Build history of the part. All positions in model axes, mm. Face numbers are marked on the shaded views. A direction names the side the tool comes from. Give positions to 0.01 mm unless a question says otherwise; leave off trailing zeros. Loops run counter-clockwise (first coordinate to the right, second up) from the corner with the lowest first, then second, coordinate; pieces in that order, holes last. Notation, with made-up numbers: (72.25, 57) -> (107.25, 57) arc R15 ccw to (107.25, 69) -> close; hole circle Ø7 at (-26, 43.5). An arc over 180 degrees is marked (long way). Answer as a JSON object with one key per item and string values. Group by question number.
Q1. Band-saw the part on B-B, the plane y = -133.5. Write the cut outline in (x, z).
Q2. Two-plate mould, pull along Y, no slides. Class the marked faces 4, 5, 6 and 7: pulls with the +Y half, pulls with the -Y half, needs draft (parallel to the pull), parting line crosses it, or undercut.
Q3. Tool access for the marked faces 1, 2 and 3: list every direction of +Z, -Z, +X, -X, +Y, -Y with a clear straight run to the whole face (end or side of a thin tool).
Q4. Drop flat-ended pins along their axis: pin 1 (16.5 mm diameter, centred on x = -8, y = 127.5, fed in from -Z); pin 2 (15.5 mm diameter, centred on x = -20, y = -64, fed in from +Z); pin 3 (1 mm diameter, centred on x = 54.5, z = 6, fed in from +Y); pin 4 (1 mm diameter, centred on x = 2.5, y = -122, fed in from -Z). Give the stop position or say it passes through.
Q5. Wall check: probe 1 along X at (y, z) = (-64, -37); probe 2 along X at (y, z) = (-64, -16.5); probe 3 along Y at (x, z) = (-20, 1). Give the ranges that are in metal, low to high. Write a range as from..to.
Q6. Band-saw the part on D-D, the plane y = 106.5. Write the cut outline in (x, z), plus the area to 3 significant figures.
Q7. Band-saw the part on A-A, the plane x = -32. Write the cut outline in (y, z).
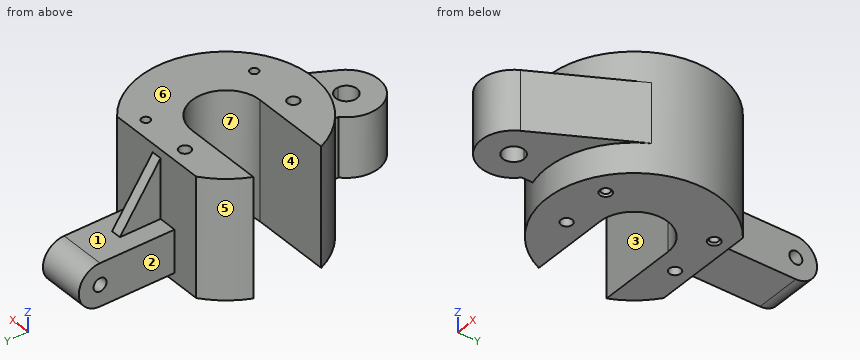
from build123d import *

# Parameters (mm, degrees)
CLAMP_BODY_PROFILE_R      = 5
CLAMP_BODY_PROFILE_R_2    = 6.75
CLAMP_BODY_DEPTH          = 70
TOP_LUG_AND_RIB_PROFILE_R = 7.668976578
TOP_LUG_DEPTH             = 27.5
GUSSET_RIB_DEPTH          = 6
BOTTOM_LUG_DEPTH          = 35
EDGE_CHAMFER_2X45_SIZE    = 2


with BuildPart() as part:
    # Clamp Body Profile → Clamp Body (new, symmetric)
    with BuildSketch(Plane.XY):
        with BuildLine():
            Line((0, -40), (-93.829632846, -40))
            ThreePointArc((-93.829632846, -40), (63.213972543, -80.04994488), (60.663003552, 82))
            Line((60.663003552, 82), (-60.663003552, 82))
            ThreePointArc((-60.663003552, 82), (-80.04994488, 63.213972543), (-93.829632846, 40))
            Line((-93.829632846, 40), (0, 40))
            ThreePointArc((0, 40), (40, 0), (0, -40))
        make_face()
        with Locations((39.991638522, 64)):
            Circle(CLAMP_BODY_PROFILE_R, mode=Mode.SUBTRACT)
        with Locations((-20, 64)):
            Circle(CLAMP_BODY_PROFILE_R_2, mode=Mode.SUBTRACT)
        with Locations(Location((39.991638522, -64, 0), (0, 0, 180))):
            Circle(CLAMP_BODY_PROFILE_R, mode=Mode.SUBTRACT)
        with Locations(Location((-20, -64, 0), (0, 0, 180))):
            Circle(CLAMP_BODY_PROFILE_R_2, mode=Mode.SUBTRACT)
    extrude(amount=CLAMP_BODY_DEPTH, both=True)

    # Top Lug and Rib Profile → Top Lug (add, symmetric)
    with BuildSketch(Plane(origin=(0, 0, 0), x_dir=(0, 0, -1), z_dir=(1, 0, 0))):
        with BuildLine():
            Line((60, 82), (60, 170))
            ThreePointArc((60, 170), (35, 195), (10, 170))
            Line((10, 170), (10, 130))
            Line((10, 130), (10, 82))
            Line((10, 82), (60, 82))
        make_face()
        with Locations((35, 170)):
            Circle(TOP_LUG_AND_RIB_PROFILE_R, mode=Mode.SUBTRACT)
    extrude(amount=TOP_LUG_DEPTH, both=True)

    # Sketch6_3 → Gusset Rib (add, symmetric)
    with BuildSketch(Plane(origin=(0, 0, 0), x_dir=(0, 0, -1), z_dir=(1, 0, 0))):
        Polygon((-60, 82), (10, 82), (10, 130), align=None)
    extrude(amount=GUSSET_RIB_DEPTH, both=True)

    # Bottom Lug Profile → Bottom Lug (add, symmetric)
    with BuildSketch(Plane.XY):
        with BuildLine():
            ThreePointArc((-27.5, -111.367680386), (-26.163106523, -169.703640044), (30.991702616, -157.947821666))
            Line((30.991702616, -157.947821666), (89.874157687, -48.235213071))
            ThreePointArc((89.874157687, -48.235213071), (51.583370989, -87.995203491), (-1.814745181, -101.983855094))
            ThreePointArc((-1.814745181, -101.983855094), (-2.152772572, -101.979344048), (-2.490826719, -101.977840326))
            Line((-2.490826719, -101.977840326), (-2.490826719, -101.969582633))
            ThreePointArc((-2.490826719, -101.969582633), (-15.1119726, -100.87431925), (-27.5, -98.222960656))
            Line((-27.5, -98.222960656), (-27.5, -111.367680386))
        make_face()
        with BuildLine():
            ThreePointArc((10.009173281, -139.977840326), (-11.329661484, -148.816675091), (-2.490826719, -127.477840326))
            ThreePointArc((-2.490826719, -127.477840326), (6.348008046, -131.139005561), (10.009173281, -139.977840326))
        make_face(mode=Mode.SUBTRACT)
    extrude(amount=BOTTOM_LUG_DEPTH, both=True)

    # Edge Chamfer 2x45
    edge_chamfer_2x45_edges = [part.edges().sort_by_distance(p)[0] for p in [
        (34.991638522, 64, -70),
        (44.991638522, -64, -70),
    ]]
    chamfer(edge_chamfer_2x45_edges, length=EDGE_CHAMFER_2X45_SIZE)


solid = part.part
Worked answers:
{
 "1": {"outline": "(-39.93, -35) -> (-13.18, -35) -> (-13.18, 35) -> (-39.93, 35) -> close; (8.2, -35) -> (44.11, -35) -> (44.11, 35) -> (8.2, 35) -> close"},
 "2": {"face 4": "undercut", "face 5": "pulls with the +Y half", "face 6": "needs draft", "face 7": "undercut"},
 "3": {"face 1": "+Z, +Y", "face 2": "+Z, -Z, -X, +Y", "face 3": "+Z, -Z, -X"},
 "4": {"pin 1": "z = -60", "pin 2": "z = 70", "pin 3": "y = 82", "pin 4": "z = -35"},
 "5": {"probe 1": "-79.42..-26.75, -13.25..34.99, 44.99..79.42", "probe 2": "-79.42..-26.75, -13.25..34.99, 44.99..81.41", "probe 3": "-173.7..-70.75, -57.25..-40, 40..57.25, 70.75..82"},
 "6": {"outline": "(-27.5, -60) -> (27.5, -60) -> (27.5, -10) -> (6, -10) -> (6, 24.27) -> (-6, 24.27) -> (-6, -10) -> (-27.5, -10) -> close", "area": "3,160 mm2"},
 "7": {"outline": "(-163.92, -35) -> (-116.04, -35) -> (-116.04, 35) -> (-163.92, 35) -> close; (-96.85, -70) -> (-40, -70) -> (-40, 70) -> (-96.85, 70) -> close; (40, -70) -> (82, -70) -> (82, 70) -> (40, 70) -> close"}
}
